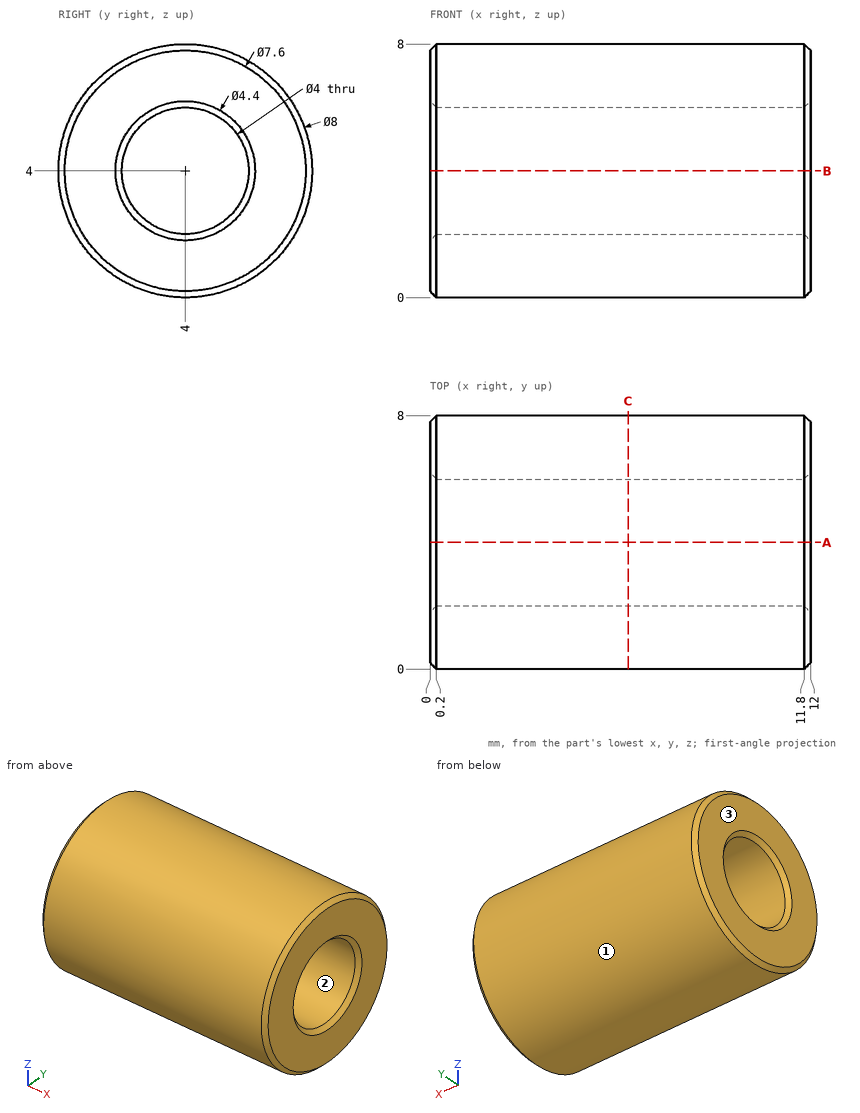
Check sheet for the drawn part. Datum: minimum x, y, z corner. Units: mm. Round coordinates to 2 decimals unless told otherwise and drop trailing zeros. Order: outer loops, then holes, each group sorted by start corner. A loop starts at its lowest first (then second) coordinate and runs counter-clockwise, first axis right, second up. Notation, with made-up numbers: (-30.75, 66) -> (-16.75, 66) arc R18 cw to (-16.75, 74) -> close; hole circle Ø10 at (-24, 1.25). An arc over 180 degrees is marked (long way). Use CSV: the item, a comma, the result in double quotes.
(1) Material ranges on line 1 along Y through (x, z) = (3.5, 4); line 2 along Z through (x, y) = (11, 5.75); line 3 along Y through (x, z) = (3.5, 3.5), recorded low to high. Write a range as from..to.
Worked out:
line 1,"0..2, 6..8"
line 2,"0.4..3.03, 4.97..7.6"
line 3,"0.03..2.06, 5.94..7.97"
(2) Depth check by flat-ended pin: pin 1 (4 mm diameter, centred on x = 5.5, z = 7, fed in from -Y). Enter the tip coordinate at first touch or a pass-through.
Worked out:
pin 1,"y = 0.13"
(3) Cross-section at C-C (x = 6.25). Record the boundary of the cut face in (y, z).
Worked out:
outline,"circle Ø8 at (4, 4); hole circle Ø4 at (4, 4)"
(4) Cross-section at A-A (y = 4). Record the boundary of the cut face in (x, z), and give its area (3 significant figures).
Worked out:
outline,"(0, 0.2) -> (0.2, 0) -> (11.8, 0) -> (12, 0.2) -> (12, 1.8) -> (11.8, 2) -> (0.2, 2) -> (0, 1.8) -> close; (0, 6.2) -> (0.2, 6) -> (11.8, 6) -> (12, 6.2) -> (12, 7.8) -> (11.8, 8) -> (0.2, 8) -> (0, 7.8) -> close"
area,"47.8 mm²"
(5) Draft check along Z on the marked faces 1, 2 and 3. Enter one of: pulls with the +Z half, pulls with the -Z half, needs draft (parallel to the pull), parting line crosses it, or undercut.
Worked out:
face 1,"parting line crosses it"
face 2,"undercut"
face 3,"needs draft"
